For this review, take the finished solid that the model builds, in its own axes (mm). A direction names the side the tool comes from. Give positions to 0.01 mm unless a question says otherwise; leave off trailing zeros. Write each loop counter-clockwise with the first axis right and the second up, starting at its lowest first coordinate (ties: lowest second). Pieces come first, ordered by that corner, then holes. Notation, with made-up numbers: M 76,60 L 83,60 A11 cw 83,79 Z; hole C 46,66.25 d9. An arc over 180 degrees is marked long. Write item = value, one per line.
```python
from build123d import *

# Parameters (mm, degrees)
SKETCH_1_W             = 20
SKETCH_1_H             = 20
EXTRUDE_1_DEPTH        = 8
HOLE_WIZARD_M4_1_D     = 3.3
HOLE_WIZARD_M4_1_DEPTH = 14.1
HOLE_WIZARD_M4_1_TIP   = 0.991420021
SKETCH_6_W             = 20
SKETCH_6_H             = 8
EXTRUDE_2_DEPTH        = 8
HOLE_WIZARD_M4_3_D     = 3.3
HOLE_WIZARD_M4_3_DEPTH = 14.1
HOLE_WIZARD_M4_3_TIP   = 0.991420021
CHAMFER_2_SIZE         = 0.5


with BuildPart() as part:
    # 草图1 → 凸台-拉伸1 (new body)
    with BuildSketch(Plane(origin=(0, 0, 0), x_dir=(1, 0, 0), z_dir=(0, 1, 0))):
        Rectangle(SKETCH_1_W, SKETCH_1_H)
    extrude(amount=EXTRUDE_1_DEPTH)

    # M4 螺纹孔1
    with Locations(Plane(origin=(10, 0, 0), x_dir=(0, 0, -1), z_dir=(1, 0, 0))):
        with Locations((5, 4), (-5, 4)):
            Hole(HOLE_WIZARD_M4_1_D / 2, depth=HOLE_WIZARD_M4_1_DEPTH)
            with Locations((0, 0, -(HOLE_WIZARD_M4_1_DEPTH + HOLE_WIZARD_M4_1_TIP / 2))):  # 118° drill point
                Cone(0, HOLE_WIZARD_M4_1_D / 2, HOLE_WIZARD_M4_1_TIP, mode=Mode.SUBTRACT)

    # 草图6 → 凸台-拉伸2 (add)
    with BuildSketch(Plane.XY.offset(10)):
        with Locations((0, -4)):
            Rectangle(SKETCH_6_W, SKETCH_6_H)
    extrude(amount=-EXTRUDE_2_DEPTH)

    # M4 螺纹孔3
    with Locations(Plane.XY.offset(10)):
        with Locations((-5, -4), (5, -4)):
            Hole(HOLE_WIZARD_M4_3_D / 2, depth=HOLE_WIZARD_M4_3_DEPTH)
            with Locations((0, 0, -(HOLE_WIZARD_M4_3_DEPTH + HOLE_WIZARD_M4_3_TIP / 2))):  # 118° drill point
                Cone(0, HOLE_WIZARD_M4_3_D / 2, HOLE_WIZARD_M4_3_TIP, mode=Mode.SUBTRACT)

    # 倒角2
    chamfer_2_edges = [part.edges().sort_by_distance(p)[0] for p in [
        (-10, 8, 0),
        (-10, 0, 10),
        (-10, -4, 2),
        (-10, 0, -4),
        (10, 4, -10),
        (0, 8, -10),
        (-10, 4, -10),
        (0, 0, -10),
        (10, -8, 6),
        (10, 0, -4),
        (10, -4, 2),
        (0, -8, 2),
        (-10, -8, 6),
        (0, -8, 10),
        (10, 8, 0),
        (0, 8, 10),
        (10, 0, 10),
    ]]
    chamfer(chamfer_2_edges, length=CHAMFER_2_SIZE)


solid = part.part
```
1. Insertion check: P1, Ø2, axis at x = -3, y = -5, coming from the -Z side; P2, Ø6, axis at x = -0.5, z = -3, coming from the -Y side; P3, Ø2, axis at y = 4, z = -5, coming from the +X side. Each pin has a flat end and moves straight along its axis. Give the tip position at first contact, or say it passes through.
Responses:
P1 = 2
P2 = 0
P3 = -4.49
2. We need section B-B, the plane y = -4. Write out the cut boundary in (x, z), then the cut area to 3 significant figures.
Responses:
outline = M -10,2.5 L -9.5,2 L -6.65,2 L -6.65,10 L -9.5,10 L -10,9.5 Z; M -3.35,2 L 3.35,2 L 3.35,10 L -3.35,10 Z; M 6.65,2 L 9.5,2 L 10,2.5 L 10,9.5 L 9.5,10 L 6.65,10 Z
area = 107 mm2
3. We need section D-D, the plane x = 0.75. Write out the cut boundary in (y, z).
Responses:
outline = M -8,2.5 L -7.5,2 L 0,2 L 0,-9.5 L 0.5,-10 L 7.5,-10 L 8,-9.5 L 8,9.5 L 7.5,10 L -7.5,10 L -8,9.5 Z; hole C 4,-5 d3.3; hole C 4,5 d3.3
4. The part is to be moulded in two halves that separate along Y. For faces 4 (the face through (2.85, 3, -6.31)), 5 (the face through (0, 4, -10)), 6 (the face through (0, 0, -4)), say which applies: +Y half, -Y half, draft (parallel to the pull), parting line (faces both ways), or undercut.
Responses:
face_4 = undercut
face_5 = draft
face_6 = -Y half
5. We need section C-C, the plane z = 0.5. Write out the cut boundary in (x, y).
Responses:
outline = M -10,0.5 L -9.5,0 L 9.5,0 L 10,0.5 L 10,7.5 L 9.5,8 L -9.5,8 L -10,7.5 Z
6. We need section A-A, the plane x = 5. Write out the cut boundary in (y, z).
Responses:
outline = M -8,2.5 L -7.5,2 L -5.65,2 L -5.65,10 L -7.5,10 L -8,9.5 Z; M -2.35,2 L 0,2 L 0,-9.5 L 0.5,-10 L 7.5,-10 L 8,-9.5 L 8,9.5 L 7.5,10 L -2.35,10 Z; hole C 4,-5 d3.3; hole C 4,5 d3.3
7. Machinability: for faces 1 (the face through (2.85, 4.07, 3.35)), 2 (the face through (0, 0, 10)), 3 (the face through (0, -4, 2)), which of the approach directions +Z, -Z, +X, -X, +Y, -Y give a long, thin tool a straight path to every point of the face, cutting with its end or side? Answer none if there is none.
Responses:
face_1 = +X
face_2 = +Z, +X, -X, +Y, -Y
face_3 = -Z, +X, -X, -Y
8. For line 1 along Y through (x, z) = (0, 5); line 2 along Y through (x, z) = (5, 5.25); line 3 along Z through (x, y) = (0.75, 5), list the stretches that pass through material, from the lowest coordinate up. Write a range as from..to.
Responses:
line_1 = -8..2.35, 5.65..8
line_2 = -8..-5.65, -2.35..2.37, 5.63..8
line_3 = -10..-6.31, -3.69..3.69, 6.31..10
